Geometry: see drawing. Coordinates: mm, zero at the bounding-box minimum. A direction names the side the tool comes from. Give positions to 0.01 mm unless a question says otherwise; leave off trailing zeros. Order: outer loops, then holes, each group sorted by start corner. A loop starts at its lowest first (then second) coordinate and runs counter-clockwise, first axis right, second up. Notation, with made-up numbers: M 31.25,85 L 49.25,85 A10 cw 49.25,95 Z; hole C -9,-15 d1. An arc over 180 degrees is marked long. Return JSON: item names as keys, results as strings.
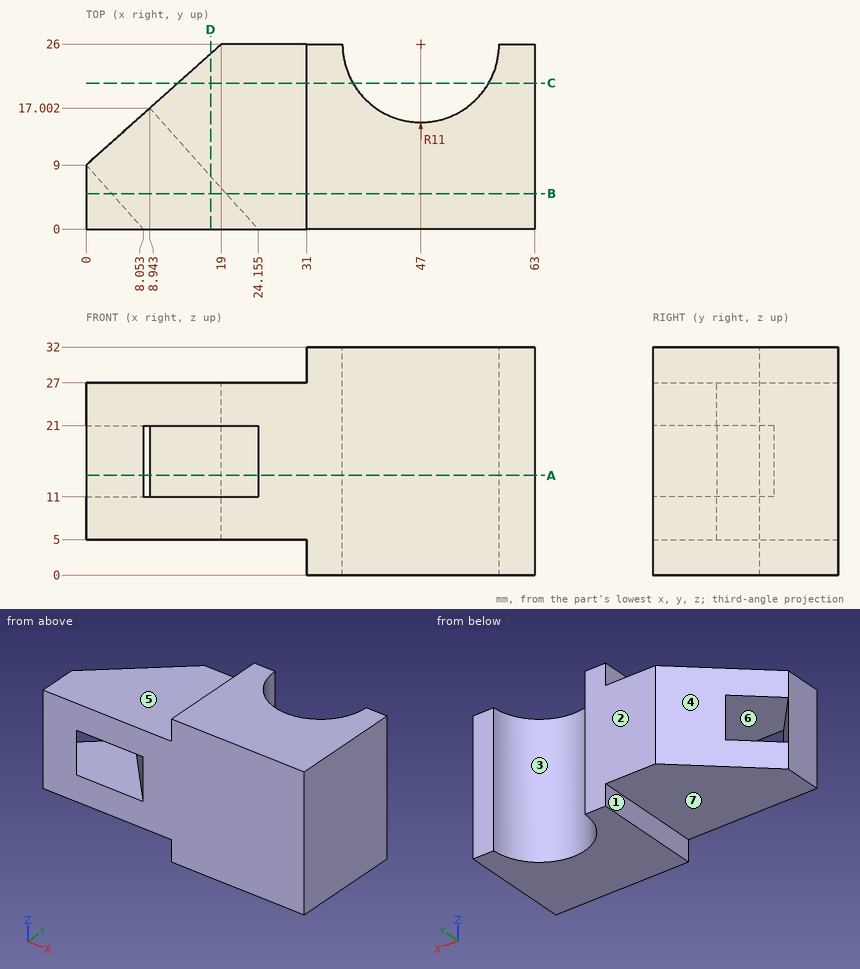
1. Ray query, probe 1 along X at (y, z) = (7.25, 4.5); probe 2 along Z at (x, y) = (21.5, 24); probe 3 along Y at (x, z) = (47, 21.5). Return the intervals inside material, ascending.
Evaluation:
{"probe 1": "x = 31 to 63", "probe 2": "z = 5 to 27", "probe 3": "y = 0 to 15"}
2. First-contact query: pin 1 (4 mm diameter, centred on y = 12, z = 1.5, fed in from -X); pin 2 (2 mm diameter, centred on y = 18, z = 22.5, fed in from -X); pin 3 (6 mm diameter, centred on y = 13.5, z = 11, fed in from -X) (1 decimal). Flat tips, straight axial feed; report the tip coordinate or a pass-through.
Evaluation:
{"pin 1": "stops at x = 31", "pin 2": "stops at x = 8.94", "pin 3": "stops at x = 1.7"}
3. Draft query along X for the marked faces 1, 2 and 3. Return one class per face: pulls with the +X half, pulls with the -X half, needs draft (parallel to the pull), parting line crosses it, or undercut.
Evaluation:
{"face 1": "pulls with the -X half", "face 2": "needs draft", "face 3": "undercut"}
4. Section query A-A (z = 14). Return loops of the section in (x, y) (1 decimal).
Evaluation:
{"outline": "M 0,0 L 8.1,0 L 0,9 Z; M 8.9,17 L 24.2,0 L 63,0 L 63,26 L 58,26 A11 cw 36,26 L 19,26 Z"}
5. Section query D-D (x = 17.5). Return loops of the section in (y, z).
Evaluation:
{"outline": "M 0,5 L 24.66,5 L 24.66,27 L 0,27 L 0,21 L 7.44,21 L 7.44,11 L 0,11 Z"}
6. Section query B-B (y = 5). Return loops of the section in (x, z), then the cut area to 4 significant figures.
Evaluation:
{"outline": "M 0,5 L 31,5 L 31,0 L 63,0 L 63,32 L 31,32 L 31,27 L 0,27 Z; hole M 3.58,11 L 19.68,11 L 19.68,21 L 3.58,21 Z", "area": "1,545 mm^2"}
7. Set-up query: the marked faces 4, 5, 6 and 7. Return all of +Z, -Z, +X, -X, +Y, -Y with unobstructed straight access to the full face (end or side cutting, diameter ignored); none if empty.
Evaluation:
{"face 4": "+Z, -Z, -X, +Y", "face 5": "+Z, -X, +Y, -Y", "face 6": "none", "face 7": "-Z, -X, +Y, -Y"}
8. Section query C-C (y = 20.5). Return loops of the section in (x, z).
Evaluation:
{"outline": "M 12.85,5 L 31,5 L 31,0 L 37.47,0 L 37.47,32 L 31,32 L 31,27 L 12.85,27 Z; M 56.53,0 L 63,0 L 63,32 L 56.53,32 Z"}
